from build123d import *

# Parameters (mm, degrees)
BASE_PLATE_DEPTH         = 30
UNDERSIDE_NOTCHES_DEPTH  = 60
PIVOT_BOSS_SKETCH_R      = 15
PIVOT_BOSS_SKETCH_R_2    = 10
PIVOT_BOSS_30_DEPTH      = 30
SLOT_RECESS_A_DEPTH      = 13
SLOT_INNER_CUT_A_DEPTH   = 5
SLOT_START               = -7
SLOT_RECESS_B_DEPTH      = 7
SLOT_INNER_CUT_B_DEPTH   = 116.758369028
BOSS_SLOT_CUT_DEPTH      = 77.811457479
BOSS_SLOT_CUT_DEPTH_BACK = 77.811457479
SUPPORT_RIB_DEPTH        = 24
RIB_TRIM_CUT_DEPTH       = 77.811457479
RIB_TRIM_CUT_DEPTH_BACK  = 77.811457479
PIVOT_BORE_SKETCH_R      = 10
PIVOT_BORE_20_DEPTH      = 48


with BuildPart() as part:
    # Base Plate Profile Sketch → Base Plate (new, symmetric)
    with BuildSketch(Plane.XY):
        Polygon((-10, 4), (10, 4), (10, 0), (50, 0), (50, 20), (-50, 20), (-50, 0), (-10, 0), align=None)
    extrude(amount=BASE_PLATE_DEPTH, both=True)

    # Underside Notches Sketch → Underside Notches (cut)
    with BuildSketch(Plane(origin=(0, 20, 0), x_dir=(1, 0, 0), z_dir=(0, 1, 0))):
        with BuildLine():
            Line((40, 30), (50, 30))
            Line((50, 30), (50, 20))
            ThreePointArc((50, 20), (47.071067812, 27.071067812), (40, 30))
        make_face()
        with BuildLine():
            Line((-50, 30), (-50, 20))
            ThreePointArc((-50, 20), (-47.071067812, 27.071067812), (-40, 30))
            Line((-40, 30), (-50, 30))
        make_face()
        with BuildLine():
            Line((-50, -30), (-50, -20))
            ThreePointArc((-50, -20), (-47.071067812, -27.071067812), (-40, -30))
            Line((-40, -30), (-50, -30))
        make_face()
        with BuildLine():
            Line((50, -30), (50, -20))
            ThreePointArc((50, -20), (47.071067812, -27.071067812), (40, -30))
            Line((40, -30), (50, -30))
        make_face()
    extrude(amount=-UNDERSIDE_NOTCHES_DEPTH, mode=Mode.SUBTRACT)

    # Pivot Boss Sketch → Pivot Boss Ø30 (add)
    with BuildSketch(Plane(origin=(0, 20, 0), x_dir=(1, 0, 0), z_dir=(0, 1, 0))):
        Circle(PIVOT_BOSS_SKETCH_R)
        with Locations(Location((0, 0, 0), (0, 0, 180))):
            Circle(PIVOT_BOSS_SKETCH_R_2, mode=Mode.SUBTRACT)
    extrude(amount=PIVOT_BOSS_30_DEPTH)

    # Slot Recess A Sketch → Slot Recess A (cut)
    with BuildSketch(Plane(origin=(0, 20, 0), x_dir=(1, 0, 0), z_dir=(0, 1, 0))):
        with BuildLine():
            Line((30, -10), (30, 10))
            ThreePointArc((30, 10), (35, 15), (40, 10))
            Line((40, 10), (40, -10))
            ThreePointArc((40, -10), (35, -15), (30, -10))
        make_face()
        with BuildLine():
            Line((-30, -10), (-30, 10))
            ThreePointArc((-30, 10), (-35, 15), (-40, 10))
            Line((-40, 10), (-40, -10))
            ThreePointArc((-40, -10), (-35, -15), (-30, -10))
        make_face()
    extrude(amount=-SLOT_RECESS_A_DEPTH, mode=Mode.SUBTRACT)

    # Slot Inner Cut A Sketch → Slot Inner Cut A (cut)
    with BuildSketch(Plane(origin=(0, 20, 0), x_dir=(1, 0, 0), z_dir=(0, 1, 0))):
        with BuildLine():
            Line((25, -10), (25, 10))
            ThreePointArc((25, 10), (35, 20), (45, 10))
            Line((45, 10), (45, -10))
            ThreePointArc((45, -10), (35, -20), (25, -10))
        make_face()
        with BuildLine():
            Line((-25, -10), (-25, 10))
            ThreePointArc((-25, 10), (-35, 20), (-45, 10))
            Line((-45, 10), (-45, -10))
            ThreePointArc((-45, -10), (-35, -20), (-25, -10))
        make_face()
    extrude(amount=-SLOT_INNER_CUT_A_DEPTH, mode=Mode.SUBTRACT)

    # Slot Recess B Sketch → Slot Recess B (cut)
    with BuildSketch(Plane.XZ.offset(SLOT_START)):
        with BuildLine():
            Line((45, 10), (45, -10))
            ThreePointArc((45, -10), (35, -20), (25, -10))
            Line((25, -10), (25, 10))
            ThreePointArc((25, 10), (35, 20), (45, 10))
        make_face()
        with BuildLine():
            Line((-45, 10), (-45, -10))
            ThreePointArc((-45, -10), (-35, -20), (-25, -10))
            Line((-25, -10), (-25, 10))
            ThreePointArc((-25, 10), (-35, 20), (-45, 10))
        make_face()
    extrude(amount=SLOT_RECESS_B_DEPTH, mode=Mode.SUBTRACT)

    # Slot Inner Cut B Sketch → Slot Inner Cut B (cut, through all)
    with BuildSketch(Plane(origin=(50, 0, 0), x_dir=(0, 0, -1), z_dir=(1, 0, 0))):
        Polygon((0, 4), (10, 4), (10, 0), (-10, 0), (-10, 4), align=None)
    extrude(amount=-SLOT_INNER_CUT_B_DEPTH, mode=Mode.SUBTRACT)

    # Boss Slot Sketch → Boss Slot Cut (cut, two sides: drawn at the far end of the back side and taken through both)
    with BuildSketch(Plane.XY.offset(-BOSS_SLOT_CUT_DEPTH_BACK)):
        Polygon((0, 50), (7, 50), (7, 40), (-7, 40), (-7, 50), align=None)
    extrude(amount=BOSS_SLOT_CUT_DEPTH + BOSS_SLOT_CUT_DEPTH_BACK, mode=Mode.SUBTRACT)

    # Support Rib Sketch → Support Rib (add, symmetric)
    with BuildSketch(Plane(origin=(0, 0, 0), x_dir=(0, 0, -1), z_dir=(1, 0, 0))):
        Polygon((0, 50), (3, 50), (3, 20), (-3, 20), (-3, 50), align=None)
    extrude(amount=SUPPORT_RIB_DEPTH, both=True)

    # Rib Trim Sketch → Rib Trim Cut (cut, two sides: drawn at the far end of the back side and taken through both)
    with BuildSketch(Plane.XY.offset(-RIB_TRIM_CUT_DEPTH_BACK)):
        Polygon((24, 20), (14.696938457, 50), (24, 50), align=None)
        Polygon((-24, 50), (-24, 20), (-14.696938457, 50), align=None)
    extrude(amount=RIB_TRIM_CUT_DEPTH + RIB_TRIM_CUT_DEPTH_BACK, mode=Mode.SUBTRACT)

    # Pivot Bore Sketch → Pivot Bore Ø20 (cut)
    with BuildSketch(Plane(origin=(0, 20, 0), x_dir=(1, 0, 0), z_dir=(0, 1, 0))):
        with Locations(Location((0, 0, 0), (0, 0, 314.427004001))):
            Circle(PIVOT_BORE_SKETCH_R)
    extrude(amount=PIVOT_BORE_20_DEPTH, mode=Mode.SUBTRACT)


solid = part.part
Work out the finished part from the listing and answer in its coordinate system (mm). A direction names the side the tool comes from. Round coordinates to 2 decimals unless told otherwise and drop trailing zeros. Order: outer loops, then holes, each group sorted by start corner. A loop starts at its lowest first (then second) coordinate and runs counter-clockwise, first axis right, second up. Notation, with made-up numbers: M 63,57.5 L 72,57.5 A20 ccw 72,87.5 Z; hole C 46,80 d10. An arc over 180 degrees is marked long. Put each result on its own line as item: value. Start each with the question number.
Q1. Flat-ended cylindrical pins translate along their axes: pin 1 (6 mm diameter, centred on x = -14, z = -22, fed in from +Y); pin 2 (6 mm diameter, centred on x = 36, z = -9.5, fed in from +Y); pin 3 (8 mm diameter, centred on y = 33, z = 4.5, fed in from +X); pin 4 (6.5 mm diameter, centred on x = -1, z = 12, fed in from +Y). Find the tip coordinate at first contact, or state that the pin passes through.
Q2. Section B-B, the plane x = -35 is taken. Write down the section's boundary in (y, z), and give its area (3 significant figures).
Q3. A tool of negligible diameter and unlimited length cuts with its end or side. For faces 1 (the flat face through (0, 40, 12)), 2 (the flat face through (-17, 2, 10)), 3 (the flat face through (-10, 2, 20)), 4 (the cylindrical face through (35, 11, -15)), 5 (the flat face through (-45, 18, 0)), from which of +Z, -Z, +X, -X, +Y, -Y can it reach the whole face along a straight path? Write none if from no direction.
Q4. Section A-A, the plane y = 5.5 is taken. Write down the section's boundary in (x, z), and give its area (3 significant figures).
Q5. Section C-C, the plane x = 0 is taken. Write down the section's boundary in (y, z), and give its area (3 significant figures).
Q6. For a pull along X with two mould halves and no side action, classify faces 6 (the flat face through (-30, 0, 22)), 7 (the cylindrical face through (35, 4, -20)), 8 (the flat face through (19.414, 34.79, -0.042)) as pulls with the +X half, pulls with the -X half, needs draft (parallel to the pull), parting line crosses it, or undercut.
Q7. Straight lines are drawn through the part: L1, parallel to X at y = 12.5, z = 9; L2, parallel to X at y = 15.5, z = 8; L3, parallel to Z at x = 0, y = 31.5. For each, find the intervals that lie inside material, in ascending order. Write a range as [from, to].
Q8. Section D-D, the plane z = 0 is taken. Give the number of separate pieces and of enclosed holes in the cut face, and give its area (3 significant figures).
Findings below:
1. pin 1: stops at y = 20
1. pin 2: passes through
1. pin 3: stops at x = 21.12
1. pin 4: stops at y = 40
2. outline: M 0,-30 L 20,-30 L 20,-20 L 15,-20 L 15,-15 L 7,-15 L 7,-20 L 0,-20 Z; M 0,20 L 7,20 L 7,15 L 15,15 L 15,20 L 20,20 L 20,30 L 0,30 Z
2. area: 480 mm^2
3. face 1: +Z, -Z, +Y
3. face 2: +X, -X, -Y
3. face 3: +Z, -Z, -Y
3. face 4: +Y, -Y
3. face 5: +Y
4. outline: M -50,-20 A10 ccw -40,-30 L 40,-30 A10 ccw 50,-20 L 50,20 A10 ccw 40,30 L -40,30 A10 ccw -50,20 Z; hole M -45,-10 A10 ccw -25,-10 L -25,10 A10 ccw -45,10 Z; hole M 25,-10 A10 ccw 45,-10 L 45,10 A10 ccw 25,10 Z
4. area: 4,490 mm^2
5. outline: M 4,-30 L 20,-30 L 20,-15 L 40,-15 L 40,-10 L 20,-10 L 20,10 L 40,10 L 40,15 L 20,15 L 20,30 L 4,30 Z
5. area: 1,160 mm^2
6. face 6: needs draft
6. face 7: undercut
6. face 8: pulls with the +X half
7. L1: x = [-50, -40], [-30, 30], [40, 50]
7. L2: x = [-50, -45], [-25, 25], [45, 50]
7. L3: z = [-15, -10], [10, 15]
8. separate pieces: 3
8. enclosed holes: 0
8. area: 1,680 mm^2
